```python
from build123d import *

# Parameters (mm, degrees)
BOSS_EXTRUDE1_DEPTH = 1.5
BOSS_EXTRUDE2_START = -1.5
SKETCH2_R           = 6
SKETCH2_R_2         = 5.1
BOSS_EXTRUDE2_DEPTH = 1
BOSS_EXTRUDE3_DEPTH = 2
SKETCH7_W           = 2
SKETCH7_H           = 19.411603012
CUT_EXTRUDE3_DEPTH  = 0.8
CUT_EXTRUDE4_START  = -1
SKETCH8_R           = 5.1
CUT_EXTRUDE4_DEPTH  = 1


with BuildPart() as part:
    # Sketch1 → Boss-Extrude1 (new body)
    with BuildSketch(Plane.XY):
        with BuildLine():
            Line((-68.5, 32.5), (68.5, 32.5))
            ThreePointArc((68.5, 32.5), (69.207106781, 32.207106781), (69.5, 31.5))
            Line((69.5, 31.5), (69.5, -31.5))
            ThreePointArc((69.5, -31.5), (69.207106781, -32.207106781), (68.5, -32.5))
            Line((68.5, -32.5), (-68.5, -32.5))
            ThreePointArc((-68.5, -32.5), (-69.207106781, -32.207106781), (-69.5, -31.5))
            Line((-69.5, -31.5), (-69.5, 31.5))
            ThreePointArc((-69.5, 31.5), (-69.207106781, 32.207106781), (-68.5, 32.5))
        make_face()
    extrude(amount=BOSS_EXTRUDE1_DEPTH)

    # Sketch2 → Boss-Extrude2 (add)
    # profile 1 of 4: a face of its own
    with BuildSketch(Plane.XY.offset(1.5).offset(BOSS_EXTRUDE2_START)):
        with Locations((-58, 18)):
            Circle(SKETCH2_R)
        with Locations((-58, 18)):
            Circle(SKETCH2_R_2, mode=Mode.SUBTRACT)
    # profile 2 of 4: a face of its own
    with BuildSketch(Plane.XY.offset(1.5).offset(BOSS_EXTRUDE2_START)):
        with Locations((58, 18)):
            Circle(SKETCH2_R)
        with Locations((58, 18)):
            Circle(SKETCH2_R_2, mode=Mode.SUBTRACT)
    # profile 3 of 4: a face of its own
    with BuildSketch(Plane.XY.offset(1.5).offset(BOSS_EXTRUDE2_START)):
        with Locations((-58, -18)):
            Circle(SKETCH2_R)
        with Locations((-58, -18)):
            Circle(SKETCH2_R_2, mode=Mode.SUBTRACT)
    # profile 4 of 4: a face of its own
    with BuildSketch(Plane.XY.offset(1.5).offset(BOSS_EXTRUDE2_START)):
        with Locations((58, -18)):
            Circle(SKETCH2_R)
        with Locations((58, -18)):
            Circle(SKETCH2_R_2, mode=Mode.SUBTRACT)
    extrude(amount=-BOSS_EXTRUDE2_DEPTH)

    # Sketch3 → Boss-Extrude3 (add)
    with BuildSketch(Plane.XY.offset(1.5)):
        with BuildLine():
            Line((60.9, 30.9), (-60.9, 30.9))
            ThreePointArc((-60.9, 30.9), (-65.849747468, 28.849747468), (-67.9, 23.9))
            Line((-67.9, 23.9), (-67.9, -23.9))
            ThreePointArc((-67.9, -23.9), (-65.849747468, -28.849747468), (-60.9, -30.9))
            Line((-60.9, -30.9), (60.9, -30.9))
            ThreePointArc((60.9, -30.9), (65.849747468, -28.849747468), (67.9, -23.9))
            Line((67.9, -23.9), (67.9, 23.9))
            ThreePointArc((67.9, 23.9), (65.849747468, 28.849747468), (60.9, 30.9))
        make_face()
        with BuildLine():
            Line((60.9, 29.3), (-60.9, 29.3))
            ThreePointArc((-60.9, 29.3), (-64.718376618, 27.718376618), (-66.3, 23.9))
            Line((-66.3, 23.9), (-66.3, -23.9))
            ThreePointArc((-66.3, -23.9), (-64.718376618, -27.718376618), (-60.9, -29.3))
            Line((-60.9, -29.3), (60.9, -29.3))
            ThreePointArc((60.9, -29.3), (64.718376618, -27.718376618), (66.3, -23.9))
            Line((66.3, -23.9), (66.3, 23.9))
            ThreePointArc((66.3, 23.9), (64.718376618, 27.718376618), (60.9, 29.3))
        make_face(mode=Mode.SUBTRACT)
    extrude(amount=BOSS_EXTRUDE3_DEPTH)

    # Sketch7 → Cut-Extrude3 (cut)
    with BuildSketch(Plane(origin=(0, -32.5, 0), x_dir=(-1, 0, 0), z_dir=(0, -1, 0))):
        Rectangle(SKETCH7_W, SKETCH7_H)
    extrude(amount=-CUT_EXTRUDE3_DEPTH, mode=Mode.SUBTRACT)

    # Sketch8 → Cut-Extrude4 (cut)
    with BuildSketch(Plane(origin=(0, 0, 0), x_dir=(-1, 0, 0), z_dir=(0, 0, -1)).offset(CUT_EXTRUDE4_START)):
        with Locations(Location((-58, 18, 0), (0, 0, 180))):
            Circle(SKETCH8_R)
        with Locations(Location((58, 18, 0), (0, 0, 180))):
            Circle(SKETCH8_R)
        with Locations(Location((58, -18, 0), (0, 0, 180))):
            Circle(SKETCH8_R)
        with Locations(Location((-58, -18, 0), (0, 0, 180))):
            Circle(SKETCH8_R)
    extrude(amount=CUT_EXTRUDE4_DEPTH, mode=Mode.SUBTRACT)


solid = part.part
```
The model under review builds one solid part; all positions refer to its coordinate system, in mm. A direction names the side the tool comes from. Round coordinates to 2 decimals unless told otherwise and drop trailing zeros. Write each loop counter-clockwise with the first axis right and the second up, starting at its lowest first coordinate (ties: lowest second). Pieces come first, ordered by that corner, then holes. Notation, with made-up numbers: (-6.75, -24) - (27.25, -24) arc R9 ccw to (27.25, -16) - close; hole circle Ø6 at (-39, 40). An arc over 180 degrees is marked (long way). Answer as CSV lines item,"result". Start each with the question number.
(1) We need section B-B on y = 18. State the section outline as (x, z) points, plus the area to 3 significant figures.
(2) Draft analysis for pull direction X (two halves, no side actions). For faces 6 (the cylindrical face through (65.8, -28.9, 2.5)), 7 (the flat face through (1, 0, 0)), 8 (the flat face through (56, 13, -1)), state which applies: pulls with the +X half, pulls with the -X half, needs draft (parallel to the pull), parting line crosses it, or undercut.
(3) We need section D-D on x = -16. State the section outline as (y, z) points, plus the area to 3 significant figures.
(4) We need section A-A on z = 2.35. State the section outline as (x, y) points.
(5) We need section C-C on x = -58. State the section outline as (y, z) points.
(6) For faces 1 (the cylindrical face through (64.76, 27.676, 2.486)), 2 (the flat face through (-60, 13, -1)), 3 (the cylindrical face through (-62.05, -21.1, 0.01)), 4 (the cylindrical face through (65.9, 28.8, 2.5)), 5 (the cylindrical face through (-65.8, 28.9, 2.5)), list the 3-axis set-ups (+Z, -Z, +X, -X, +Y, -Y) from which the entire face can be reached by the end or side of a thin tool; tool diameter is ignored.
(7) To check wall thickness, follow line 1 (Y direction, x = 58, z = -0.2); line 2 (Y direction, x = -58, z = 0.05); line 3 (X direction, y = -18, z = 0.2). State the ranges of each line that lie inside material, in increasing order.
(8) For pin 1 Ø3 at (x, y) = (-58.5, 17) entering from -Z; pin 2 Ø0.6 at (y, z) = (10.5, 3) entering from +X; pin 3 Ø8 at (x, y) = (-17.5, 9) entering from +Z, all flat-tipped, find the tip position at first contact; note any pin that passes through.
Worked answers:
1,outline,"(-69.5, 0) - (-64, 0) - (-64, -1) - (-63.1, -1) - (-63.1, 1) - (-52.9, 1) - (-52.9, -1) - (-52, -1) - (-52, 0) - (52, 0) - (52, -1) - (52.9, -1) - (52.9, 1) - (63.1, 1) - (63.1, -1) - (64, -1) - (64, 0) - (69.5, 0) - (69.5, 1.5) - (67.9, 1.5) - (67.9, 3.5) - (66.3, 3.5) - (66.3, 1.5) - (-66.3, 1.5) - (-66.3, 3.5) - (-67.9, 3.5) - (-67.9, 1.5) - (-69.5, 1.5) - close"
1,area,"198 mm²"
2,face 6,"pulls with the +X half"
2,face 7,"undercut"
2,face 8,"needs draft"
3,outline,"(-32.5, 0) - (32.5, 0) - (32.5, 1.5) - (30.9, 1.5) - (30.9, 3.5) - (29.3, 3.5) - (29.3, 1.5) - (-29.3, 1.5) - (-29.3, 3.5) - (-30.9, 3.5) - (-30.9, 1.5) - (-32.5, 1.5) - close"
3,area,"104 mm²"
4,outline,"(-67.9, -23.9) arc R7 ccw to (-60.9, -30.9) - (60.9, -30.9) arc R7 ccw to (67.9, -23.9) - (67.9, 23.9) arc R7 ccw to (60.9, 30.9) - (-60.9, 30.9) arc R7 ccw to (-67.9, 23.9) - close; hole (-66.3, -23.9) arc R5.4 ccw to (-60.9, -29.3) - (60.9, -29.3) arc R5.4 ccw to (66.3, -23.9) - (66.3, 23.9) arc R5.4 ccw to (60.9, 29.3) - (-60.9, 29.3) arc R5.4 ccw to (-66.3, 23.9) - close"
5,outline,"(-32.5, 0) - (-24, 0) - (-24, -1) - (-23.1, -1) - (-23.1, 1) - (-12.9, 1) - (-12.9, -1) - (-12, -1) - (-12, 0) - (12, 0) - (12, -1) - (12.9, -1) - (12.9, 1) - (23.1, 1) - (23.1, -1) - (24, -1) - (24, 0) - (32.5, 0) - (32.5, 1.5) - (30.9, 1.5) - (30.9, 3.5) - (29.3, 3.5) - (29.3, 1.5) - (-29.3, 1.5) - (-29.3, 3.5) - (-30.9, 3.5) - (-30.9, 1.5) - (-32.5, 1.5) - close"
6,face 1,"+Z"
6,face 2,"-Z, +X, -X, +Y, -Y"
6,face 3,"-Z"
6,face 4,"+Z, +X, +Y"
6,face 5,"+Z, -X, +Y"
7,line 1,"-24 to -23.1, -12.9 to -12, 12 to 12.9, 23.1 to 24"
7,line 2,"-32.5 to -23.1, -12.9 to 12.9, 23.1 to 32.5"
7,line 3,"-69.5 to -63.1, -52.9 to 52.9, 63.1 to 69.5"
8,pin 1,"z = 1"
8,pin 2,"x = 67.9"
8,pin 3,"z = 1.5"
